from build123d import *

# Parameters (mm, degrees)
SKETCH1_R           = 5.5
SKETCH1_W           = 20.2
SKETCH1_H           = 14.2
BOSS_EXTRUDE1_DEPTH = 10


with BuildPart() as part:
    # Sketch1 → Boss-Extrude1 (new body)
    with BuildSketch(Plane.XY):
        with BuildLine():
            Line((538.108108788, 869.539360157), (628.108108788, 816.518490855))
            ThreePointArc((628.108108788, 816.518490855), (631.692997782, 812.867012092), (633.002234094, 807.920232682))
            Line((633.002234094, 807.920232682), (633.002234094, 573.941101984))
            ThreePointArc((633.002234094, 573.941101984), (630.659088344, 568.284247734), (625.002234094, 565.941101984))
            Line((625.002234094, 565.941101984), (567.061111031, 565.941101984))
            Line((567.061111031, 565.941101984), (567.061111031, 560.941101984))
            Line((567.061111031, 560.941101984), (549.061111031, 560.941101984))
            Line((549.061111031, 560.941101984), (549.061111031, 565.941101984))
            Line((549.061111031, 565.941101984), (332.061111031, 565.941101984))
            Line((332.061111031, 565.941101984), (332.061111031, 560.941101984))
            Line((332.061111031, 560.941101984), (314.061111031, 560.941101984))
            Line((314.061111031, 560.941101984), (314.061111031, 565.941101984))
            Line((314.061111031, 565.941101984), (271.002234094, 565.941101984))
            ThreePointArc((271.002234094, 565.941101984), (265.345379845, 568.284247734), (263.002234094, 573.941101984))
            Line((263.002234094, 573.941101984), (263.002234094, 702.941101984))
            Line((263.002234094, 702.941101984), (303.002234094, 702.941101984))
            ThreePointArc((303.002234094, 702.941101984), (310.073301906, 705.870034172), (313.002234094, 712.941101984))
            Line((313.002234094, 712.941101984), (313.002234094, 752.941101984))
            ThreePointArc((313.002234094, 752.941101984), (310.073301906, 760.012169796), (303.002234094, 762.941101984))
            Line((303.002234094, 762.941101984), (263.002234094, 762.941101984))
            Line((263.002234094, 762.941101984), (263.002234094, 862.941101984))
            ThreePointArc((263.002234094, 862.941101984), (265.345379845, 868.597956233), (271.002234094, 870.941101984))
            Line((271.002234094, 870.941101984), (533.002234094, 870.941101984))
            ThreePointArc((533.002234094, 870.941101984), (535.649630765, 870.584301187), (538.108108788, 869.539360157))
        make_face()
        with Locations((358.002234094, 683.941101984)):
            Circle(SKETCH1_R, mode=Mode.SUBTRACT)
        with Locations((294.102234094, 633.241101984)):
            Rectangle(SKETCH1_W, SKETCH1_H, mode=Mode.SUBTRACT)
        with Locations((434.102234094, 633.241101984)):
            Rectangle(SKETCH1_W, SKETCH1_H, mode=Mode.SUBTRACT)
        with Locations((294.102234094, 813.041101984)):
            Rectangle(SKETCH1_W, SKETCH1_H, mode=Mode.SUBTRACT)
        with Locations((434.102234094, 813.041101984)):
            Rectangle(SKETCH1_W, SKETCH1_H, mode=Mode.SUBTRACT)
    extrude(amount=BOSS_EXTRUDE1_DEPTH)


solid = part.part
Could you check a few things on this model? Use its own coordinates, in mm. A direction names the side the tool comes from. Coordinates: 2 decimals unless noted, no trailing zeros. Order: outer loops, then holes, each group sorted by start corner. A loop starts at its lowest first (then second) coordinate and runs counter-clockwise, first axis right, second up.
Q1. Suppose I cut it at A-A on z = 7.5. Give the number of separate pieces and of enclosed holes in the cut face, and give its area (3 significant figures).
Q2. Suppose I cut it at B-B on x = 506. Please give me the cut outline in (y, z).
Q3. Which directions (+Z, -Z, +X, -X, +Y, -Y) give clear straight access to the entire face, cutting with the end or side of a thin tool? Please do faces 4 (the flat face through (304.202, 813, 5)), 5 (the flat face through (263.002, 812, 5)), 6 (the cylindrical face through (310, 705.8, 4.9)).
Q4. Thinking about a two-plate mould opening in X: for faces 1 (the flat face through (294, 805.941, 5)), 2 (the flat face through (582.48, 843.4, 4.93)), 3 (the flat face through (263.002, 638, 5)), which applies, released by +X, released by -X, zero draft, split by the parting line, or undercut?
Q5. Please list where these lines run through material, in increasing order: L1, parallel to X at y = 810, z = 8; L2, parallel to Y at x = 413.5, z = 7; L3, parallel to X at y = 729.5, z = 9.75.
Q6. Will these pins go through, and if not, where does the flat tip stop? pin 1 (6 mm diameter, centred on x = 553, z = 5.5, fed in from +Y); pin 2 (4 mm diameter, centred on y = 562.5, z = 7, fed in from +X); pin 3 (5 mm diameter, centred on y = 735.5, z = 7, fed in from -X); pin 4 (1.5 mm diameter, centred on x = 386.5, y = 653.5, fed in from -Z).
Q7. Suppose I cut it at C-C on y = 832. Please give me the cut outline in (x, z), and give its area (3 significant figures).
Answer:
1. separate pieces: 1
1. enclosed holes: 5
1. area: 106,000 mm2
2. outline: (565.94, 0) - (870.94, 0) - (870.94, 10) - (565.94, 10) - close
3. face 4: +Z, -Z
3. face 5: +Z, -Z, -X, +Y, -Y
3. face 6: +Z, -Z, -X
4. face 1: undercut
4. face 2: released by +X
4. face 3: released by -X
5. L1: x = 263 to 284, 304.2 to 424, 444.2 to 632.78
5. L2: y = 565.94 to 870.94
5. L3: x = 313 to 633
6. pin 1: stops at y = 862.53
6. pin 2: stops at x = 567.06
6. pin 3: stops at x = 313
6. pin 4: stops at z = 0
7. outline: (263, 0) - (601.83, 0) - (601.83, 10) - (263, 10) - close
7. area: 3,390 mm2
